from build123d import *

# Parameters (mm, degrees)
SKETCH_1_W                   = 540
SKETCH_1_H                   = 40
EXTRUDE_1_DEPTH              = 12
CHAMFER_1_SIZE               = 2
F_4_0MM_1_D                  = 4
F_4_0MM_1_DEPTH              = 12
F_4_0MM_1_TIP                = 1.201721238
PATTERN_LINEAR_4_COUNT       = 9
PATTERN_LINEAR_4_PITCH       = 60
HOLE_WIZARD_M6_1_D           = 6.6
HOLE_WIZARD_M6_1_CBORE_D     = 11
HOLE_WIZARD_M6_1_CBORE_DEPTH = 6.8
PATTERN_LINEAR_5_COUNT       = 8
PATTERN_LINEAR_5_PITCH       = 60


with BuildPart() as part:
    # 草图1 → 凸台-拉伸1 (new body)
    with BuildSketch(Plane(origin=(0, 0, 0), x_dir=(1, 0, 0), z_dir=(0, 1, 0))):
        Rectangle(SKETCH_1_W, SKETCH_1_H)
    extrude(amount=EXTRUDE_1_DEPTH)

    # 倒角1
    chamfer_1_edges = [part.edges().sort_by_distance(p)[0] for p in [
        (270, 6, 20),
        (-270, 6, 20),
        (-270, 6, -20),
        (270, 6, -20),
    ]]
    chamfer(chamfer_1_edges, length=CHAMFER_1_SIZE)

    # Ø4.0mm 暗销孔1
    with Locations(Plane(origin=(0, 0, 0), x_dir=(-1, 0, 0), z_dir=(0, -1, 0))):
        with Locations((-240, 9.5), (240, 9.5)):
            Hole(F_4_0MM_1_D / 2, depth=F_4_0MM_1_DEPTH)
            with Locations((0, 0, -(F_4_0MM_1_DEPTH + F_4_0MM_1_TIP / 2))):  # 118° drill point
                Cone(0, F_4_0MM_1_D / 2, F_4_0MM_1_TIP, mode=Mode.SUBTRACT)

    # 草图6 → M3 螺纹孔1 (revolve, cut)
    with BuildSketch(Plane(origin=(240, 0, 0), x_dir=(0, 0, -1), z_dir=(1, 0, 0))):
        Polygon((0, 0), (0, 8.251075774), (1.25, 7.5), (1.25, 0), align=None)
    hole_wizard_m3_1 = revolve(axis=Axis((240, -6.35, 0), (0, 1, 0)), mode=Mode.SUBTRACT)

    # 阵列(线性)4: M3 螺纹孔1 ×9
    with Locations(*[(-i * PATTERN_LINEAR_4_PITCH, 0, 0) for i in range(1, PATTERN_LINEAR_4_COUNT)]):
        add(hole_wizard_m3_1, mode=Mode.SUBTRACT)

    # M6 六角圆柱头螺钉的柱形沉头孔1 (through all)
    with Locations(Plane(origin=(0, 0, 0), x_dir=(-1, 0, 0), z_dir=(0, -1, 0))):
        with Locations((210, 0)):
            hole_wizard_m6_1 = CounterBoreHole(HOLE_WIZARD_M6_1_D / 2, HOLE_WIZARD_M6_1_CBORE_D / 2, HOLE_WIZARD_M6_1_CBORE_DEPTH)

    # 阵列(线性)5: M6 六角圆柱头螺钉的柱形沉头孔1 ×8
    with Locations(*[(i * PATTERN_LINEAR_5_PITCH, 0, 0) for i in range(1, PATTERN_LINEAR_5_COUNT)]):
        add(hole_wizard_m6_1, mode=Mode.SUBTRACT)


solid = part.part
Build history of the part. All positions in model axes, mm. A direction names the side the tool comes from. Round coordinates to 2 decimals unless told otherwise and drop trailing zeros. One line per question, with ' | ' between items.
1. Mould opens along Z. For faces 1 (the face through (150, 6.8, 4)), 2 (the face through (-4, 6, 20)), 3 (the face through (-94, 6.8, 0)), 4 (the face through (-4, 0, 0)) say: released by +Z, released by -Z, zero draft, split by the parting line, or undercut.
Results are:
face 1: undercut | face 2: released by +Z | face 3: undercut | face 4: zero draft
2. Tool access for faces 5 (the face through (35.495, 3.352, -0.242)), 6 (the face through (-4, 12, 0)): list every direction of +Z, -Z, +X, -X, +Y, -Y with a clear straight run to the whole face (end or side of a thin tool).
Results are:
face 5: -Y | face 6: +Z, -Z, +X, -X, +Y
3. Drop flat-ended pins along their axis: pin 1 Ø1 at (x, z) = (36, -6) entering from -Y; pin 2 Ø10 at (x, z) = (-30, 0) entering from -Y; pin 3 Ø6 at (x, z) = (-210, 0) entering from -Y. Give the stop position or say it passes through.
Results are:
pin 1: y = 0 | pin 2: y = 6.8 | pin 3: through
4. Band-saw the part on A-A, the plane y = 2.5. Give the number of separate pieces and of enclosed holes in the cut face, and give its area (3 significant figures).
Results are:
separate pieces: 1 | enclosed holes: 19 | area: 20,800 mm^2
5. Drill centre lines: line 1 along X through (y, z) = (9.75, -11); line 2 along Z through (x, y) = (30, 9.8); line 3 along Z through (x, y) = (-151, 4.25). Where is each one in solid material? Low to high. Write a range as from..to.
Results are:
line 1: -270..-241.32, -238.68..238.68, 241.32..270 | line 2: -20..-3.3, 3.3..20 | line 3: -20..-5.41, 5.41..20
